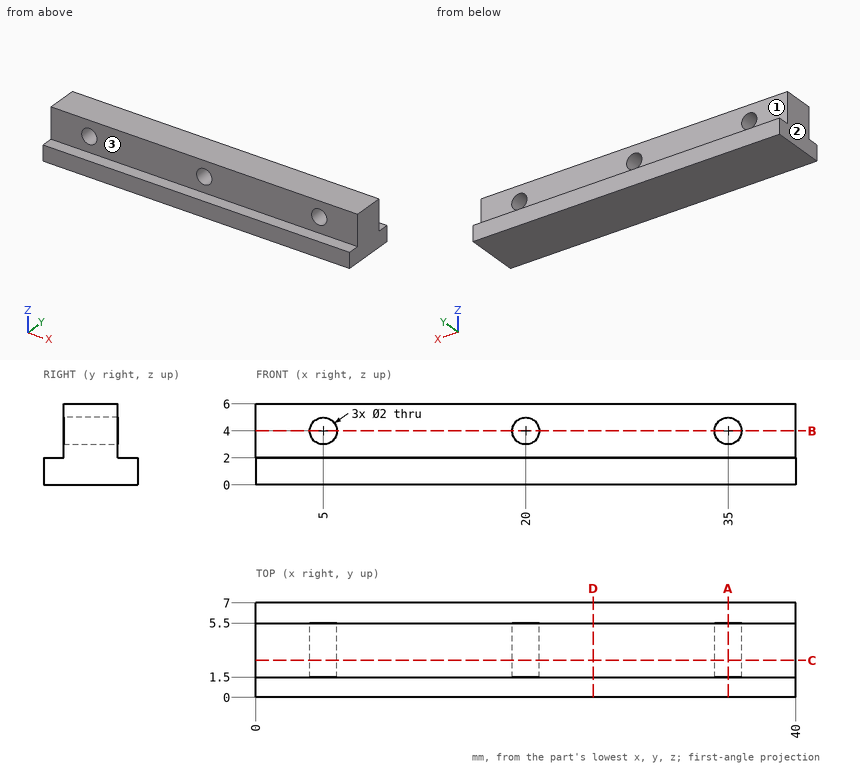
Verification items for this drawing (mm, ordinates from the low corner). A direction names the side the tool comes from. Give positions to 0.01 mm unless a question says otherwise; leave off trailing zeros. Write each loop counter-clockwise with the first axis right and the second up, starting at its lowest first coordinate (ties: lowest second). Pieces come first, ordered by that corner, then holes. Notation, with made-up numbers: (-32.75, 38) -> (-12.75, 38) arc R20 ccw to (-12.75, 63) -> close; hole circle Ø3 at (21.5, 40). An arc over 180 degrees is marked (long way). Use CSV: the item, a comma, the result in double quotes.
(1) Set-up check for the marked faces 1, 2 and 3: record each of +Z, -Z, +X, -X, +Y, -Y from which the full face is reachable in a straight line by a thin tool's end or side.
Derived:
face 1,"+Z, +X, -X, +Y"
face 2,"+Z, -Z, -X, +Y, -Y"
face 3,"+Z, +X, -X, -Y"
(2) Sectioned sample at B-B (z = 4). Record the cut outline in (x, y).
Derived:
outline,"(0, 1.5) -> (4, 1.5) -> (4, 5.5) -> (0, 5.5) -> close; (6, 1.5) -> (19, 1.5) -> (19, 5.5) -> (6, 5.5) -> close; (21, 1.5) -> (34, 1.5) -> (34, 5.5) -> (21, 5.5) -> close; (36, 1.5) -> (40, 1.5) -> (40, 5.5) -> (36, 5.5) -> close"
(3) Sectioned sample at C-C (y = 2.75). Record the cut outline in (x, z).
Derived:
outline,"(0, 0) -> (40, 0) -> (40, 6) -> (0, 6) -> close; hole circle Ø2 at (5, 4); hole circle Ø2 at (20, 4); hole circle Ø2 at (35, 4)"
(4) Go/stop test with flat-tipped pins: pin 1 (1.5 mm diameter, centred on x = 36, z = 4.5, fed in from +Y); pin 2 (1.6 mm diameter, centred on x = 13, y = 6, fed in from +Z); pin 3 (1.8 mm diameter, centred on x = 5, z = 4, fed in from -Y); pin 4 (2 mm diameter, centred on x = 14.5, z = 4.5, fed in from -Y). Record where each tip stops, or that it passes through.
Derived:
pin 1,"stops at y = 5.5"
pin 2,"stops at z = 6"
pin 3,"passes through"
pin 4,"stops at y = 1.5"
(5) Sectioned sample at A-A (x = 35). Record the cut outline in (y, z).
Derived:
outline,"(0, 0) -> (7, 0) -> (7, 2) -> (5.5, 2) -> (5.5, 3) -> (1.5, 3) -> (1.5, 2) -> (0, 2) -> close; (1.5, 5) -> (5.5, 5) -> (5.5, 6) -> (1.5, 6) -> close"
(6) Material ranges on L1, parallel to X at y = 2.75, z = 4; L2, parallel to Z at x = 35, y = 2; L3, parallel to X at y = 3, z = 4.85, recorded low to high.
Derived:
L1,"x = 0 to 4, 6 to 19, 21 to 34, 36 to 40"
L2,"z = 0 to 3, 5 to 6"
L3,"x = 0 to 4.47, 5.53 to 19.47, 20.53 to 34.47, 35.53 to 40"
(7) Sectioned sample at D-D (x = 25). Record the cut outline in (y, z).
Derived:
outline,"(0, 0) -> (7, 0) -> (7, 2) -> (5.5, 2) -> (5.5, 6) -> (1.5, 6) -> (1.5, 2) -> (0, 2) -> close"
